The listing builds one solid part. Answer for the finished solid, in the listing's coordinates (mm). Give positions to 0.01 mm unless a question says otherwise; leave off trailing zeros. Write each loop counter-clockwise with the first axis right and the second up, starting at its lowest first coordinate (ties: lowest second). Pieces come first, ordered by that corner, then holes. Notation, with made-up numbers: (-10, 13) - (24, 13) arc R12 ccw to (24, 32) - close; hole circle Ø9 at (-10, 10). An arc over 180 degrees is marked (long way). Write each question's results on one line, items separated by ' | '. Start each with the question number.
Q1. Section C-C (x = 8.25) is taken. Determine the outline of the cut face in (y, z), plus the area to 4 significant figures.
Q2. Section A-A (y = 4.25) is taken. Determine the outline of the cut face in (x, z).
Q3. Find the intervals of material crossed by probe 1 along X at (y, z) = (3.6, 70.5); probe 2 along Y at (x, z) = (7.5, 70), in increasing order.
Q4. Section B-B (z = 149) is taken. Determine the outline of the cut face in (x, y).
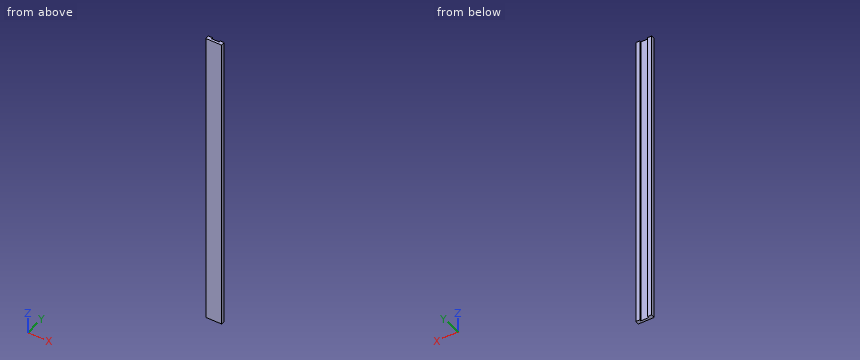
```python
from build123d import *

# Parameters (mm, degrees)
BOSS_EXTRUDE1_DEPTH = 385


with BuildPart() as part:
    # Sketch1 → Boss-Extrude1 (new body)
    with BuildSketch(Plane.XY):
        Polygon((5, 5), (5, 3), (15, 3), (15, 5), (20, 5), (20, 0), (0, 0), (0, 5), align=None)
    extrude(amount=BOSS_EXTRUDE1_DEPTH)


solid = part.part
```
Answers below:
1) outline: (0, 0) - (3, 0) - (3, 385) - (0, 385) - close | area: 1,155 mm2
2) outline: (0, 0) - (5, 0) - (5, 385) - (0, 385) - close; (15, 0) - (20, 0) - (20, 385) - (15, 385) - close
3) probe 1: x = 0 to 5, 15 to 20 | probe 2: y = 0 to 3
4) outline: (0, 0) - (20, 0) - (20, 5) - (15, 5) - (15, 3) - (5, 3) - (5, 5) - (0, 5) - close
